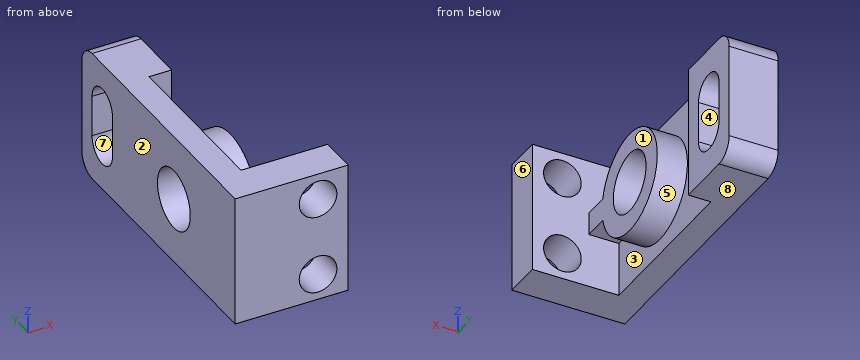
```python
from build123d import *

# Parameters (mm, degrees)
L_BRACKET_BODY_DEPTH     = 17.5
UPRIGHT_TOP_FILLETS_R5_R = 5
BASE_HOLES_REACH         = 75.697
BASE_HOLES_SKETCH_R      = 5
PIVOT_BOSS_SKETCH_R      = 8
PIVOT_BOSS_DEPTH         = 8
PIVOT_BORE_REACH         = 82.376
SKETCH5_2_R              = 8
TOP_SLOT_REACH           = 80.869


with BuildPart() as part:
    # L Bracket Profile Sketch → L Bracket Body (new, symmetric)
    with BuildSketch(Plane.XY):
        Polygon((0, 0), (0, 75), (13, 75), (13, 55), (7, 55), (7, 10), (30, 10), (30, 0), align=None)
    extrude(amount=L_BRACKET_BODY_DEPTH, both=True)

    # Upright Top Fillets R5
    upright_top_fillets_r5_edges = [part.edges().sort_by_distance(p)[0] for p in [
        (6.5, 75, 17.5),
        (6.5, 75, -17.5),
    ]]
    fillet(upright_top_fillets_r5_edges, radius=UPRIGHT_TOP_FILLETS_R5_R)

    # Base Holes Sketch → Base Holes (cut, up to next)
    with BuildSketch(Plane(origin=(0, 10, 0), x_dir=(1, 0, 0), z_dir=(0, 1, 0)), mode=Mode.PRIVATE) as base_holes_sk1:
        with Locations(Location((22, -10.5, 0), (0, 0, 270))):
            Circle(BASE_HOLES_SKETCH_R)
    base_holes_tool1 = extrude(base_holes_sk1.sketch, amount=-BASE_HOLES_REACH, mode=Mode.PRIVATE) & part.part
    # Base Holes Sketch → Base Holes (cut, up to next)
    with BuildSketch(Plane(origin=(0, 10, 0), x_dir=(1, 0, 0), z_dir=(0, 1, 0)), mode=Mode.PRIVATE) as base_holes_sk2:
        with Locations(Location((22, 10.5, 0), (0, 0, 270))):
            Circle(BASE_HOLES_SKETCH_R)
    base_holes_tool2 = extrude(base_holes_sk2.sketch, amount=-BASE_HOLES_REACH, mode=Mode.PRIVATE) & part.part
    add(base_holes_tool1.solids().sort_by_distance((22, 10, 10.5))[0], mode=Mode.SUBTRACT)
    add(base_holes_tool2.solids().sort_by_distance((22, 10, -10.5))[0], mode=Mode.SUBTRACT)

    # Pivot Boss Sketch → Pivot Boss (add)
    with BuildSketch(Plane(origin=(7, 0, 0), x_dir=(0, 0, -1), z_dir=(1, 0, 0))):
        with BuildLine():
            Line((3, 16.837553419), (3, 10))
            Line((3, 10), (-3, 10))
            Line((-3, 10), (-3, 16.837553419))
            ThreePointArc((-3, 16.837553419), (0, 43.5), (3, 16.837553419))
        make_face()
        with Locations(Location((0, 30, 0), (0, 0, 90))):
            Circle(PIVOT_BOSS_SKETCH_R, mode=Mode.SUBTRACT)
    extrude(amount=PIVOT_BOSS_DEPTH)

    # Sketch5_2 → Pivot Bore (cut, up to next)
    with BuildSketch(Plane(origin=(7, 0, 0), x_dir=(0, 0, -1), z_dir=(1, 0, 0)), mode=Mode.PRIVATE) as pivot_bore_sk1:
        with Locations(Location((0, 30, 0), (0, 0, 90))):
            Circle(SKETCH5_2_R)
    pivot_bore_tool1 = extrude(pivot_bore_sk1.sketch, amount=-PIVOT_BORE_REACH, mode=Mode.PRIVATE) & part.part
    add(pivot_bore_tool1.solids().sort_by_distance((7, 30, 0))[0], mode=Mode.SUBTRACT)

    # Top Slot Sketch → Top Slot (cut, up to next)
    with BuildSketch(Plane(origin=(13, 0, 0), x_dir=(0, 0, -1), z_dir=(1, 0, 0)), mode=Mode.PRIVATE) as top_slot_sk1:
        with BuildLine():
            Line((-5.5, 70), (5.5, 70))
            ThreePointArc((5.5, 70), (10.5, 65), (5.5, 60))
            Line((5.5, 60), (-5.5, 60))
            ThreePointArc((-5.5, 60), (-10.5, 65), (-5.5, 70))
        make_face()
    top_slot_tool1 = extrude(top_slot_sk1.sketch, amount=-TOP_SLOT_REACH, mode=Mode.PRIVATE) & part.part
    add(top_slot_tool1.solids().sort_by_distance((13, 65, 0))[0], mode=Mode.SUBTRACT)


solid = part.part
```
Geometry: final body of the model. Coordinates: model frame, mm. Face numbers are marked on the shaded views. A direction names the side the tool comes from. Coordinates: 2 decimals unless noted, no trailing zeros. Order: outer loops, then holes, each group sorted by start corner. A loop starts at its lowest first (then second) coordinate and runs counter-clockwise, first axis right, second up. Notation, with made-up numbers: (16, 63) -> (71, 63) arc R13 cw to (71, 72) -> close; hole circle Ø3 at (-32.5, 7.5). An arc over 180 degrees is marked (long way). Answer in a Markdown table with one row per item.
Item 1: Section C-C on y = 65. Output: boundary loops of the cut face in (x, z), plus the area to 3 significant figures.
Return value:
| item | result |
|---|---|
| outline | (0, -17.5) -> (13, -17.5) -> (13, -10.5) -> (0, -10.5) -> close; (0, 10.5) -> (13, 10.5) -> (13, 17.5) -> (0, 17.5) -> close |
| area | 182 mm² |
Item 2: Contact query for flat-ended pins moving along their axis: P1, Ø3, axis at x = 11, z = -5.5, coming from the -Y side; P2, Ø21, axis at y = 30, z = 0, coming from the +X side; P3, Ø3.5, axis at x = 11.5, y = 13.5, coming from the -Z side; P4, Ø6, axis at x = 22, z = 10.5, coming from the +Y side. Output: stop coordinate, or through.
Return value:
| item | result |
|---|---|
| P1 | stops at y = 0 |
| P2 | stops at x = 15 |
| P3 | stops at z = -3 |
| P4 | passes through |
Item 3: Ray query, L1, parallel to Z at x = 10.75, y = 30; L2, parallel to Z at x = 21.5, y = 5; L3, parallel to X at y = 43, z = -13. Return the intervals inside material, ascending.
Return value:
| item | result |
|---|---|
| L1 | z = -13.5 to -8, 8 to 13.5 |
| L2 | z = -17.5 to -15.47, -5.53 to 5.53, 15.47 to 17.5 |
| L3 | x = 0 to 7 |
Item 4: Draft query along Z for the marked faces 5, 6, 7 and 8. Return one class per face: released by +Z, released by -Z, zero draft, split by the parting line, or undercut.
Return value:
| item | result |
|---|---|
| face 5 | split by the parting line |
| face 6 | zero draft |
| face 7 | undercut |
| face 8 | released by -Z |
Item 5: Section A-A on x = 12.25. Output: boundary loops of the cut face in (y, z), plus the area to 3 significant figures.
Return value:
| item | result |
|---|---|
| outline | (0, -17.5) -> (10, -17.5) -> (10, -3) -> (16.84, -3) arc R13.5 ccw (long way) to (16.84, 3) -> (10, 3) -> (10, 17.5) -> (0, 17.5) -> close; (55, -17.5) -> (70, -17.5) arc R5 ccw to (75, -12.5) -> (75, 12.5) arc R5 ccw to (70, 17.5) -> (55, 17.5) -> close; hole circle Ø16 at (30, 0); hole (60, -5.5) arc R5 ccw to (70, -5.5) -> (70, 5.5) arc R5 ccw to (60, 5.5) -> close |
| area | 1,260 mm² |
Item 6: Section D-D on y = 9. Output: boundary loops of the cut face in (x, z), plus the area to 3 significant figures.
Return value:
| item | result |
|---|---|
| outline | (0, -17.5) -> (30, -17.5) -> (30, 17.5) -> (0, 17.5) -> close; hole circle Ø10 at (22, -10.5); hole circle Ø10 at (22, 10.5) |
| area | 893 mm² |
Item 7: Access query for the marked faces 1, 2, 3 and 4. Directions: +Z, -Z, +X, -X, +Y, -Y. A direction counts if a zero-diameter tool reaches every point of the face in a straight line with its end or side. Return the directions, or none.
Return value:
| item | result |
|---|---|
| face 1 | +Z, -Z, +X, +Y |
| face 2 | +Z, -Z, -X, +Y, -Y |
| face 3 | +X |
| face 4 | +X, -X |
Item 8: Section B-B on x = 22. Output: boundary loops of the cut face in (y, z), plus the area to 3 significant figures.
Return value:
| item | result |
|---|---|
| outline | (0, -17.5) -> (10, -17.5) -> (10, -15.5) -> (0, -15.5) -> close; (0, -5.5) -> (10, -5.5) -> (10, 5.5) -> (0, 5.5) -> close; (0, 15.5) -> (10, 15.5) -> (10, 17.5) -> (0, 17.5) -> close |
| area | 150 mm² |
